Can you work these out from the model? Positions are in its coordinate system, mm. Round coordinates to 2 decimals unless told otherwise and drop trailing zeros. Write each loop counter-clockwise with the first axis right and the second up, starting at its lowest first coordinate (ties: lowest second). Pieces come first, ordered by that corner, then holes. Notation, with made-up numbers: (39.5, 76.25) - (45.5, 76.25) arc R11 ccw to (45.5, 89.25) - close; hole circle Ø5 at (69.25, -5). An arc over 180 degrees is marked (long way). One line per item, written item: value. Start each with the question number.
(1) I want a section at D-D on z = 30. List the corners of the cut face in (x, y) for me.
(2) I want a section at B-B on y = 0. List the corners of the cut face in (x, z) for me.
(3) Thinking about a two-plate mould opening in X: for faces 1 (the face through (-3, -3, 0)), 2 (the face through (1.138, -0.056, 38.726)), 3 (the face through (-3.695, 1.532, 20.46)), which applies, +X half, -X half, draft (parallel to the pull), parting line (faces both ways), or undercut?
(4) I want a section at A-A on x = 0. List the corners of the cut face in (y, z) for me, plus the area to 3 significant figures.
(5) I want a section at C-C on z = 38. List the corners of the cut face in (x, y) for me, plus the area to 3 significant figures.
(6) If I drill on L1, parallel to Z at x = 0, y = -0.75; L2, parallel to Z at x = 5.25, y = -1.25; L3, parallel to X at y = 2.25, z = 38, over which ranges is the centre line in solid material (lowest first)? Write a range as from..to.
(7) I'm going to push flat-ended pins straight in: pin 1 Ø1 at (x, z) = (-0.5, 18) entering from +Y; pin 2 Ø2 at (x, y) = (1, 4.5) entering from +Z; pin 3 Ø8 at (y, z) = (2.5, 30) entering from +X. Where does each tip first touch, or does it pass through?
from build123d import *

# Parameters (mm, degrees)
SKETCH1_R               = 4
BOSS_EXTRUDE1_DEPTH     = 42
SKETCH2_R               = 7.5
BOSS_EXTRUDE2_DEPTH     = 4
CUT_EXTRUDE1_DEPTH      = 44.318587235
CUT_EXTRUDE1_DEPTH_BACK = 44.318587235
SKETCH3_R               = 1.35
CHAMFER1_SIZE           = 0.5


with BuildPart() as part:
    # Sketch1 → Boss-Extrude1 (new body)
    with BuildSketch(Plane.XY):
        with Locations(Location((0, 0, 0), (0, 0, 180))):
            Circle(SKETCH1_R)
    extrude(amount=BOSS_EXTRUDE1_DEPTH)

    # Sketch2 → Boss-Extrude2 (add)
    with BuildSketch(Plane(origin=(0, 0, 0), x_dir=(-1, 0, 0), z_dir=(0, 0, -1))):
        Circle(SKETCH2_R)
    extrude(amount=BOSS_EXTRUDE2_DEPTH)

    # Sketch3 → Cut-Extrude1 (cut, two sides: drawn at the far end of the back side and taken through both)
    with BuildSketch(Plane(origin=(0, 0, 0), x_dir=(1, 0, 0), z_dir=(0, 1, 0)).offset(-CUT_EXTRUDE1_DEPTH_BACK)):
        with Locations(Location((0, -38, 0), (0, 0, 270))):
            Circle(SKETCH3_R)
    extrude(amount=CUT_EXTRUDE1_DEPTH + CUT_EXTRUDE1_DEPTH_BACK, mode=Mode.SUBTRACT)

    # Chamfer1
    chamfer1_edges = [part.edges().sort_by_distance(p)[0] for p in [
        (4, 0, 42),
        (7.5, 0, 0),
        (7.5, 0, -4),
    ]]
    chamfer(chamfer1_edges, length=CHAMFER1_SIZE)


solid = part.part
Established:
1. outline: circle Ø8 at (0, 0)
2. outline: (-7.5, -3.5) - (-7, -4) - (7, -4) - (7.5, -3.5) - (7.5, -0.5) - (7, 0) - (4, 0) - (4, 41.5) - (3.5, 42) - (-3.5, 42) - (-4, 41.5) - (-4, 0) - (-7, 0) - (-7.5, -0.5) - close; hole circle Ø2.7 at (0, 38)
3. face 1: draft
3. face 2: undercut
3. face 3: parting line
4. outline: (-7.5, -3.5) - (-7, -4) - (7, -4) - (7.5, -3.5) - (7.5, -0.5) - (7, 0) - (4, 0) - (4, 36.65) - (-4, 36.65) - (-4, 0) - (-7, 0) - (-7.5, -0.5) - close; (-4, 39.35) - (4, 39.35) - (4, 41.5) - (3.5, 42) - (-3.5, 42) - (-4, 41.5) - close
4. area: 374 mm2
5. outline: (-1.35, -3.77) - (-1.35, 3.77) arc R4 ccw to start; (1.35, -3.77) arc R4 ccw to (1.35, 3.77) - close
5. area: 29.1 mm2
6. L1: -4..36.65, 39.35..42
6. L2: -4..0
6. L3: -3.31..-1.35, 1.35..3.31
7. pin 1: y = 4
7. pin 2: z = 41.89
7. pin 3: x = 4
